Geometry check sheet. Reference: drawing and pictorial views, mm from the part's lowest x, y, z. Give positions to 0.01 mm unless a question says otherwise; leave off trailing zeros. Loops run counter-clockwise (first coordinate to the right, second up) from the corner with the lowest first, then second, coordinate; pieces in that order, holes last. Notation, with made-up numbers: (24.25, -38.5) - (72.25, -38.5) arc R20 cw to (72.25, -14.5) - close; hole circle Ø1 at (84.25, 34.5). An arc over 180 degrees is marked (long way). Answer in a Markdown table with one row per item. Add a question column.
(1) Sectioned sample at C-C on z = 1. State how many separate pieces and enclosed holes the cut face has, then the cut area to 3 significant figures.
(2) Sectioned sample at A-A on x = 65. Enter the section's corners in (y, z).
(3) Sectioned sample at B-B on y = 125. Enter the section's corners in (x, z).
(4) Thickness scan on L1, parallel to X at y = 53, z = 0.85; L2, parallel to X at y = 34.5, z = 0.75 (1 decimal); L3, parallel to Y at x = 65, z = 1.2. Record the ranges inside material, lowest first.
(5) Sectioned sample at D-D on y = 95. Enter the section's corners in (x, z).
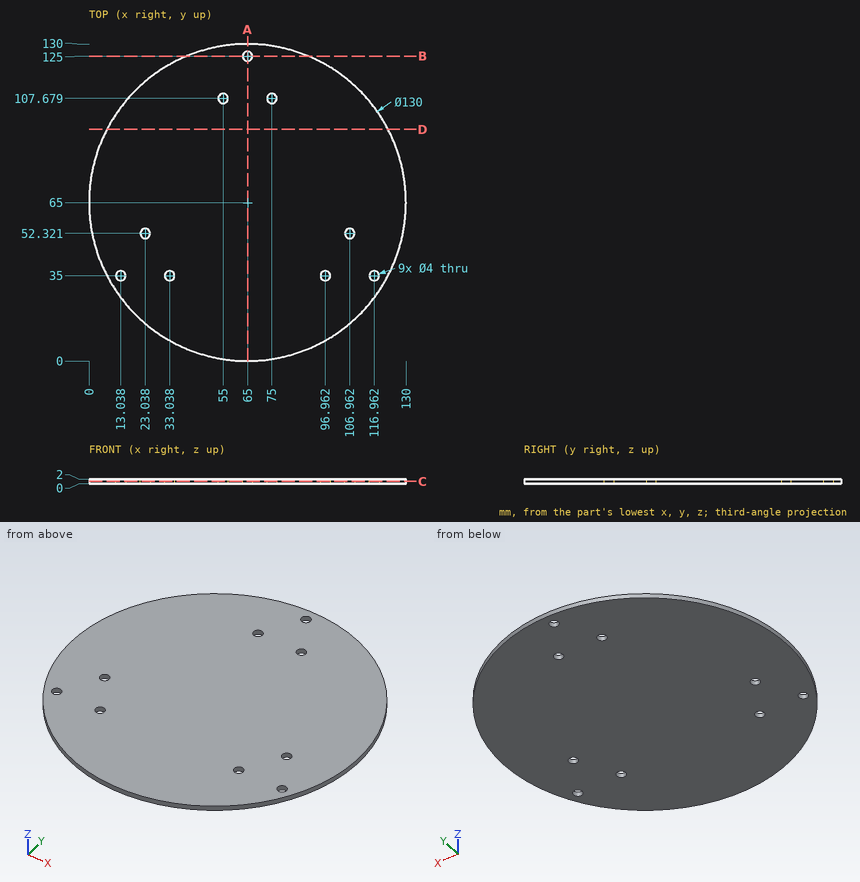
Reply:
| question | item | result |
|---|---|---|
| 1 | separate pieces | 1 |
| 1 | enclosed holes | 9 |
| 1 | area | 13,200 mm^2 |
| 2 | outline | (0, 0) - (123, 0) - (123, 2) - (0, 2) - close; (127, 0) - (130, 0) - (130, 2) - (127, 2) - close |
| 3 | outline | (40, 0) - (63, 0) - (63, 2) - (40, 2) - close; (67, 0) - (90, 0) - (90, 2) - (67, 2) - close |
| 4 | L1 | 1.12 to 21.16, 24.92 to 105.08, 108.84 to 128.88 |
| 4 | L2 | 7.6 to 11.1, 15 to 31.1, 35 to 95, 98.9 to 115, 118.9 to 122.4 |
| 4 | L3 | 0 to 123, 127 to 130 |
| 5 | outline | (7.34, 0) - (122.66, 0) - (122.66, 2) - (7.34, 2) - close |
